The model under review builds one solid part; all positions refer to its coordinate system, in mm. A direction names the side the tool comes from. Round coordinates to 2 decimals unless told otherwise and drop trailing zeros. Write each loop counter-clockwise with the first axis right and the second up, starting at its lowest first coordinate (ties: lowest second). Pieces come first, ordered by that corner, then holes. Notation, with made-up numbers: M -32,87.25 L -13,87.25 A21 ccw -13,113.25 Z; hole C 30,64 d3. An arc over 180 degrees is marked long. One line per item, written item: value. Start each with the question number.
1) Take a section at A-A, the plane z = 28. Write out the cut boundary in (x, y), and give its area (3 significant figures).
2) Tool access review of faces 1 (the face through (-6.453, -11.24, 0.266)), 2 (the face through (6.2, -5.4, 10)): name each direction out of +Z, -Z, +X, -X, +Y, -Y from which nothing blocks a thin tool from reaching the whole face with its end or side.
3) For P1, Ø3, axis at x = -6.5, z = 60.5, coming from the -Y side (3 decimals); P2, Ø2, axis at y = -6, z = 16, coming from the +X side (3 decimals); P3, Ø5, axis at x = 5, z = 42.5, coming from the -Y side; P4, Ø10, axis at x = -1.5, y = -1, coming from the -Z side, all flat-tipped, find the tip position at first contact; note any pin that passes through.
4) Wall thickness on probe 1 along Y at (x, z) = (0, 11); probe 2 along Z at (x, y) = (11.75, -2.75); probe 3 along Y at (x, z) = (2, 38): over which ranges is each line inside the solid? List them lowest first.
from build123d import *

# Parameters (mm, degrees)
HEX_HEAD_25AF_X10_DEPTH        = 10
HEAD_CHAMFER_PROFILE_OUTSIDE_W = 73.404
HEAD_CHAMFER_PROFILE_OUTSIDE_H = 69.536
HEAD_CHAMFER_PROFILE_OUTSIDE_R = 12.5
HEAD_CHAMFER_CUT_DEPTH         = 10
HEAD_CHAMFER_CUT_DRAFT         = -60
SHANK_PROFILE_16_R             = 8
SHANK_16_X68_DEPTH             = 68


with BuildPart() as part:
    # Hex Head Profile 25AF → Hex Head 25AF x10 (new body)
    with BuildSketch(Plane.XY):
        Polygon((14.43375673, 0), (7.216878365, 12.5), (-7.216878365, 12.5), (-14.43375673, 0), (-7.216878365, -12.5), (7.216878365, -12.5), align=None)
    extrude(amount=HEX_HEAD_25AF_X10_DEPTH)


with BuildPart() as head_chamfer_cut_tool:
    # Head Chamfer Profile outside → Head Chamfer Cut (with draft: the straight prism first)
    with BuildSketch(Plane(origin=(0, 0, 0), x_dir=(-1, 0, 0), z_dir=(0, 0, -1))):
        Rectangle(HEAD_CHAMFER_PROFILE_OUTSIDE_W, HEAD_CHAMFER_PROFILE_OUTSIDE_H)
        Circle(HEAD_CHAMFER_PROFILE_OUTSIDE_R, mode=Mode.SUBTRACT)
    extrude(amount=-HEAD_CHAMFER_CUT_DEPTH)
    # Head Chamfer Cut: the draft: its side faces are tilted about the plane it starts from
    head_chamfer_cut_sides = [head_chamfer_cut_tool.faces().sort_by_distance(p)[0] for p in [
        (0, -34.768, 5),
        (-36.702, 0, 5),
        (0, 34.768, 5),
        (36.702, 0, 5),
        (12.5, 0, 5),
    ]]
    draft(head_chamfer_cut_sides, Plane(origin=(0, 0, 0), x_dir=(-1, 0, 0), z_dir=(0, 0, -1)), HEAD_CHAMFER_CUT_DRAFT)


with BuildPart() as part_1:
    add(part.part)

    # Head Chamfer Cut: cut by head_chamfer_cut_tool
    add(head_chamfer_cut_tool.part, mode=Mode.SUBTRACT)

    # Shank Profile Ø16 → Shank Ø16 x68 (add)
    with BuildSketch(Plane.XY.offset(10)):
        Circle(SHANK_PROFILE_16_R)
    extrude(amount=SHANK_16_X68_DEPTH)


solid = part_1.part
Checked values:
1. outline: C 0,0 d16
1. area: 201 mm2
2. face 1: -Z, -X, -Y
2. face 2: +Z
3. P1: stops at y = -6.245
3. P2: stops at x = 6.245
3. P3: stops at y = -7.6
3. P4: stops at z = 0
4. probe 1: y = -8 to 8
4. probe 2: z = 0 to 10
4. probe 3: y = -7.75 to 7.75
